CAD build for the part. Positions are in the model's coordinates, mm. Coordinates: 2 decimals unless noted, no trailing zeros. Loops run counter-clockwise (first coordinate to the right, second up) from the corner with the lowest first, then second, coordinate; pieces in that order, holes last. Notation, with made-up numbers: M 11.5,51 L 46.5,51 A27 cw 46.5,73 Z; hole C 69.25,83 d5. An arc over 180 degrees is marked long. Answer as a JSON object with one key per item and string values. Group by question number.
```python
from build123d import *

# Parameters (mm, degrees)
SKETCH_1_W      = 82.2
SKETCH_1_H      = 9
EXTRUDE_1_DEPTH = 1.5
FILLET_1_R      = 0.5
FILLET_2_R      = 1


with BuildPart() as part:
    # 草图1 → 凸台-拉伸1 (new body)
    with BuildSketch(Plane(origin=(0, 0, 0), x_dir=(1, 0, 0), z_dir=(0, 1, 0))):
        with BuildLine():
            Line((44.1, 7), (-44.1, 7))
            Line((-44.1, 7), (-44.1, 4.2))
            ThreePointArc((-44.1, 4.2), (-43.5, 3.6), (-44.1, 3))
            Line((-44.1, 3), (-46.6, 3))
            Line((-46.6, 3), (-46.6, -3))
            Line((-46.6, -3), (-44.1, -3))
            ThreePointArc((-44.1, -3), (-43.5, -3.6), (-44.1, -4.2))
            Line((-44.1, -4.2), (-44.1, -7))
            Line((-44.1, -7), (44.1, -7))
            Line((44.1, -7), (44.1, -4.2))
            ThreePointArc((44.1, -4.2), (43.5, -3.6), (44.1, -3))
            Line((44.1, -3), (46.6, -3))
            Line((46.6, -3), (46.6, 3))
            Line((46.6, 3), (44.1, 3))
            ThreePointArc((44.1, 3), (43.5, 3.6), (44.1, 4.2))
            Line((44.1, 4.2), (44.1, 7))
        make_face()
        Rectangle(SKETCH_1_W, SKETCH_1_H, mode=Mode.SUBTRACT)
    extrude(amount=EXTRUDE_1_DEPTH)

    # 圆角1
    fillet_1_edges = [part.edges().sort_by_distance(p)[0] for p in [
        (46.6, 0.75, -3),
        (46.6, 0.75, 3),
        (-46.6, 0.75, 3),
        (-46.6, 0.75, -3),
    ]]
    fillet(fillet_1_edges, radius=FILLET_1_R)

    # 圆角2
    fillet_2_edges = [part.edges().sort_by_distance(p)[0] for p in [
        (-44.1, 0.75, -7),
        (44.1, 0.75, -7),
        (44.1, 0.75, 7),
        (-44.1, 0.75, 7),
        (-41.1, 0.75, -4.5),
        (-41.1, 0.75, 4.5),
        (41.1, 0.75, 4.5),
        (41.1, 0.75, -4.5),
    ]]
    fillet(fillet_2_edges, radius=FILLET_2_R)


solid = part.part
```
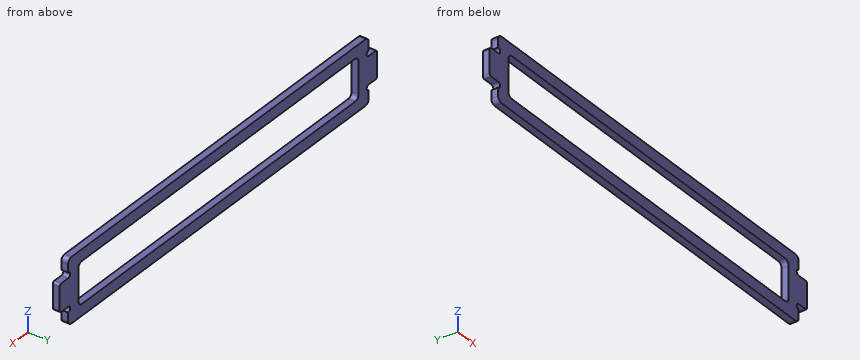
Item 1: Pin check, flat tip, straight feed: pin 1 (0.8 mm diameter, centred on x = -45.5, y = 0.5, fed in from +Z). Stop position of the tip, or through.
Item 2: Slice it at A-A, the plane x = -26. Write the cut outline in (y, z), then the cut area to 3 significant figures.
Item 3: Drill centre lines: L1, parallel to Z at x = 24.5, y = 0.9; L2, parallel to X at y = 0.45, z = -0.75; L3, parallel to X at y = 0.4, z = 5. Where is each one in solid material? Low to high. Write a range as from..to.
Computed:
{
 "1": {"pin 1": "z = 3"},
 "2": {"outline": "M 0,-7 L 1.5,-7 L 1.5,-4.5 L 0,-4.5 Z; M 0,4.5 L 1.5,4.5 L 1.5,7 L 0,7 Z", "area": "7.50 mm2"},
 "3": {"L1": "-7..-4.5, 4.5..7", "L2": "-46.6..-41.1, 41.1..46.6", "L3": "-44.1..44.1"}
}
